```python
from build123d import *

# Parameters (mm, degrees)
PLATE_PROFILE_SKETCH_R   = 1.778
PLATE_PROFILE_SKETCH_R_2 = 2.54
PLATE_BODY_0_12IN_DEPTH  = 3.048
FILLETS_R0_12IN_R        = 3.048


with BuildPart() as part:
    # Plate Profile Sketch → Plate Body 0.12in (new body)
    with BuildSketch(Plane.XY):
        with BuildLine():
            Line((-19.05, 5.08), (-24.886815787, 5.08))
            ThreePointArc((-24.886815787, 5.08), (0, 25.4), (24.886815787, 5.08))
            Line((24.886815787, 5.08), (19.05, 5.08))
            ThreePointArc((19.05, 5.08), (13.97, 0), (19.05, -5.08))
            Line((19.05, -5.08), (24.886815787, -5.08))
            ThreePointArc((24.886815787, -5.08), (0, -25.4), (-24.886815787, -5.08))
            Line((-24.886815787, -5.08), (-19.05, -5.08))
            ThreePointArc((-19.05, -5.08), (-13.97, 0), (-19.05, 5.08))
        make_face()
        with Locations(Location((0, 19.05, 0), (0, 0, 180))):
            Circle(PLATE_PROFILE_SKETCH_R, mode=Mode.SUBTRACT)
        with Locations(Location((0, -19.05, 0), (0, 0, 180))):
            Circle(PLATE_PROFILE_SKETCH_R, mode=Mode.SUBTRACT)
        with Locations(Location((0, 0, 0), (0, 0, 180))):
            Circle(PLATE_PROFILE_SKETCH_R_2, mode=Mode.SUBTRACT)
    extrude(amount=PLATE_BODY_0_12IN_DEPTH)

    # Fillets R0.12in
    fillets_r0_12in_edges = [part.edges().sort_by_distance(p)[0] for p in [
        (-24.886815787, 5.08, 1.524),
        (24.886815787, 5.08, 1.524),
        (24.886815787, -5.08, 1.524),
        (-24.886815787, -5.08, 1.524),
    ]]
    fillet(fillets_r0_12in_edges, radius=FILLETS_R0_12IN_R)


solid = part.part
```
Geometry: final body of the model. Coordinates: model frame, mm. A direction names the side the tool comes from. Coordinates: 2 decimals unless noted, no trailing zeros. Order: outer loops, then holes, each group sorted by start corner. A loop starts at its lowest first (then second) coordinate and runs counter-clockwise, first axis right, second up.
Item 1: Material intervals for line 1 along X through (y, z) = (19.05, 1.3); line 2 along X through (y, z) = (19, 2.15); line 3 along Y through (x, z) = (18, 1.4), sorted ascending.
Answer:
line 1: x = -16.8 to -1.78, 1.78 to 16.8
line 2: x = -16.86 to -1.78, 1.78 to 16.86
line 3: y = -17.92 to -4.97, 4.97 to 17.92
Item 2: Draft query along Y for faces 4 (the face through (0.33, -2.52, 1.5)), 5 (the face through (-5, 0, 3.048)), 6 (the face through (-0.426, 25.396, 1.503)), 7 (the face through (13.97, 0.11, 1.5)). Return one class per face: released by +Y, released by -Y, zero draft, split by the parting line, or undercut.
Answer:
face 4: undercut
face 5: zero draft
face 6: released by +Y
face 7: undercut
Item 3: Contact query for flat-ended pins moving along their axis: P1, Ø5.5, axis at x = 0, y = 19.05, coming from the +Z side; P2, Ø0.5, axis at x = -20.5, z = 2, coming from the +Y side; P3, Ø0.9, axis at x = 19.5, z = 1, coming from the -Y side. Output: stop coordinate, or through.
Answer:
P1: stops at z = 3.05
P2: stops at y = 15.33
P3: stops at y = -16.8
Item 4: Access query for faces 1 (the face through (-20, 5.08, 2)), 2 (the face through (20, 5.08, 2)), 3 (the face through (-5, 0, 0)). Directions: +Z, -Z, +X, -X, +Y, -Y. A direction counts if a zero-diameter tool reaches every point of the face in a straight line with its end or side. Return the directions, or none.
Answer:
face 1: +Z, -Z, -X
face 2: +Z, -Z, +X
face 3: -Z, +X, -X, +Y, -Y
Item 5: Section query B-B (x = 0). Output: boundary loops of the cut face in (y, z), then the cut area to 3 significant figures.
Answer:
outline: (-25.4, 0) - (-20.83, 0) - (-20.83, 3.05) - (-25.4, 3.05) - close; (-17.27, 0) - (-2.54, 0) - (-2.54, 3.05) - (-17.27, 3.05) - close; (2.54, 0) - (17.27, 0) - (17.27, 3.05) - (2.54, 3.05) - close; (20.83, 0) - (25.4, 0) - (25.4, 3.05) - (20.83, 3.05) - close
area: 118 mm2
Item 6: Section query D-D (y = 19.05). Output: boundary loops of the cut face in (x, z), then the cut area to 3 significant figures.
Answer:
outline: (-16.8, 0) - (-1.78, 0) - (-1.78, 3.05) - (-16.8, 3.05) - close; (1.78, 0) - (16.8, 0) - (16.8, 3.05) - (1.78, 3.05) - close
area: 91.6 mm2
Item 7: Section query C-C (y = 0). Output: boundary loops of the cut face in (x, z), then the cut area to 3 significant figures.
Answer:
outline: (-13.97, 0) - (-2.54, 0) - (-2.54, 3.05) - (-13.97, 3.05) - close; (2.54, 0) - (13.97, 0) - (13.97, 3.05) - (2.54, 3.05) - close
area: 69.7 mm2
Item 8: Section query A-A (z = 1.5). Output: boundary loops of the cut face in (x, y), then the cut area to 3 significant figures.
Answer:
outline: (-23.66, -9.24) arc R25.4 ccw to (23.66, -9.24) arc R3.05 ccw to (20.82, -5.08) - (19.05, -5.08) arc R5.08 cw to (19.05, 5.08) - (20.82, 5.08) arc R3.05 ccw to (23.66, 9.24) arc R25.4 ccw to (-23.66, 9.24) arc R3.05 ccw to (-20.82, 5.08) - (-19.05, 5.08) arc R5.08 cw to (-19.05, -5.08) - (-20.82, -5.08) arc R3.05 ccw to start; hole circle Ø5.08 at (0, 0); hole circle Ø3.56 at (0, -19.05); hole circle Ø3.56 at (0, 19.05)
area: 1,760 mm2
